```python
from build123d import *

# Parameters (mm, degrees)
BOSS_EXTRUDE1_DEPTH = 220
SHELL1_T            = -2
CUT_EXTRUDE1_DEPTH  = 321.212491043
SKETCH3_R           = 2.5
CUT_EXTRUDE2_DEPTH  = 394.612153142
SKETCH4_W           = 120
SKETCH4_H           = 120
CUT_EXTRUDE3_DEPTH  = 376.254580252
CUT_EXTRUDE4_DEPTH  = 120
FILLET1_R           = 10
CUT_EXTRUDE5_REACH  = 377.255
SKETCH6_W           = 20
SKETCH6_H           = 25
CUT_EXTRUDE6_DEPTH  = 25
FILLET2_R           = 5
SKETCH8_W           = 20
SKETCH8_H           = 52
CUT_EXTRUDE7_DEPTH  = 357.766015962
CUT_EXTRUDE8_DEPTH  = 20
FILLET3_R           = 5


with BuildPart() as part:
    # Sketch1 → Boss-Extrude1 (new body)
    with BuildSketch(Plane.XY):
        Polygon((-164.523614444, 0), (-116.335763439, -116.335763439), (0, -164.523614444), (116.335763439, -116.335763439), (164.523614444, 0), (116.335763439, 116.335763439), (0, 164.523614444), (-116.335763439, 116.335763439), align=None)
    extrude(amount=BOSS_EXTRUDE1_DEPTH)

    # Shell1
    shell1_openings = [part.faces().sort_by_distance(p)[0] for p in [
        (0, 0, 220),
        (0, 0, 0),
    ]]
    offset(amount=SHELL1_T, openings=shell1_openings, kind=Kind.INTERSECTION)

    # Sketch2 → Cut-Extrude1 (cut, through all)
    with BuildSketch(Plane.XY.offset(220)):
        Polygon((75.61693775, 182.555436661), (-82.042454152, -198.068005503), (95.714298716, -271.697263345), (253.373690618, 108.92617882), align=None)
    extrude(amount=-CUT_EXTRUDE1_DEPTH, mode=Mode.SUBTRACT)

    # Sketch3 → Cut-Extrude2 (cut, through all)
    with BuildSketch(Plane(origin=(-58.167881719, -140.429688942, 0), x_dir=(0.9238795325112961, -0.3826834323650676, 0), z_dir=(-0.3826834323650675, -0.923879532511296, 0))):
        with Locations((-12, 200)):
            Circle(SKETCH3_R)
        with Locations((-12, 140)):
            Circle(SKETCH3_R)
        with Locations((-12, 80)):
            Circle(SKETCH3_R)
    extrude(amount=-CUT_EXTRUDE2_DEPTH, mode=Mode.SUBTRACT)

    # Sketch4 → Cut-Extrude3 (cut, through all)
    with BuildSketch(Plane(origin=(-58.167881719, 140.429688942, 0), x_dir=(0.9238795325112777, 0.3826834323651116, 0), z_dir=(-0.38268343236511165, 0.9238795325112779, 0))):
        with Locations((12.039538519, -60)):
            Rectangle(SKETCH4_W, SKETCH4_H)
    extrude(amount=-CUT_EXTRUDE3_DEPTH, mode=Mode.SUBTRACT)

    # Sketch5 → Cut-Extrude4 (cut)
    with BuildSketch(Plane(origin=(0, 0, 0), x_dir=(-1, 0, 0), z_dir=(0, 0, -1))):
        Polygon((-12.944778014, 156.996927428), (-11.862385814, 159.610053358), (-13.710144879, 158.844686494), align=None)
    extrude(amount=-CUT_EXTRUDE4_DEPTH, mode=Mode.SUBTRACT)

    # Fillet1
    fillet1_edges = [part.edges().sort_by_distance(p)[0] for p in [
        (-102.094887019, 121.152135392, 120),
        (13.327461447, 157.920806961, 120),
    ]]
    fillet(fillet1_edges, radius=FILLET1_R)

    # Sketch6 → Cut-Extrude5 (cut, up to next)
    with BuildSketch(Plane(origin=(-58.167881719, 140.429688942, 0), x_dir=(0.9238795325112777, 0.3826834323651116, 0), z_dir=(-0.38268343236511165, 0.9238795325112779, 0)), mode=Mode.PRIVATE) as cut_extrude5_sk1:
        with Locations((-57.960461481, -12.5)):
            Rectangle(SKETCH6_W, SKETCH6_H)
    cut_extrude5_tool1 = extrude(cut_extrude5_sk1.sketch, amount=-CUT_EXTRUDE5_REACH, mode=Mode.PRIVATE) & part.part
    add(cut_extrude5_tool1.solids().sort_by_distance((-111.716366, 118.249181, 12.5))[0], mode=Mode.SUBTRACT)

    # Sketch7 → Cut-Extrude6 (cut)
    with BuildSketch(Plane(origin=(0, 0, 0), x_dir=(-1, 0, 0), z_dir=(0, 0, -1))):
        Polygon((117.959351739, 107.189822685), (119.04174394, 109.802948615), (119.807110804, 107.95518955), align=None)
    extrude(amount=-CUT_EXTRUDE6_DEPTH, mode=Mode.SUBTRACT)

    # Fillet2
    fillet2_edges = [part.edges().sort_by_distance(p)[0] for p in [
        (-118.883231272, 107.572506117, 25),
    ]]
    fillet(fillet2_edges, radius=FILLET2_R)

    # Sketch8 → Cut-Extrude7 (cut, through all)
    with BuildSketch(Plane(origin=(-140.429688942, 58.167881719, 0), x_dir=(0, 0, 1), z_dir=(-0.9238795325112957, 0.3826834323650681, 0))):
        with Locations((10, -40.960461481)):
            Rectangle(SKETCH8_W, SKETCH8_H)
    extrude(amount=-CUT_EXTRUDE7_DEPTH, mode=Mode.SUBTRACT)

    # Sketch9 → Cut-Extrude8 (cut)
    with BuildSketch(Plane(origin=(0, 0, 0), x_dir=(-1, 0, 0), z_dir=(0, 0, -1))):
        Polygon((159.745704114, -6.30864406), (161.593463179, -7.074010925), (162.358830044, -5.22625186), align=None)
    extrude(amount=-CUT_EXTRUDE8_DEPTH, mode=Mode.SUBTRACT)

    # Fillet3
    fillet3_edges = [part.edges().sort_by_distance(p)[0] for p in [
        (-145.230930158, 43.963534128, 20),
        (-160.669583647, -6.691327492, 20),
    ]]
    fillet(fillet3_edges, radius=FILLET3_R)


solid = part.part
```
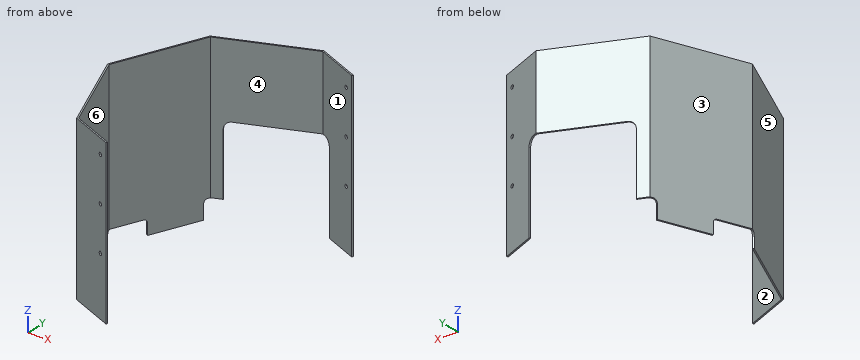
Work out the finished part from the listing and answer in its coordinate system (mm). Face numbers are marked on the shaded views. A direction names the side the tool comes from. Round coordinates to 2 decimals unless told otherwise and drop trailing zeros. Order: outer loops, then holes, each group sorted by start corner. A loop starts at its lowest first (then second) coordinate and runs counter-clockwise, first axis right, second up.
Q1. A cutting plane is placed at D-D, the plane y = -79.5. Determine the outline of the cut face in (x, z).
Solution:
outline: (-131.59, 0) - (-129.43, 0) - (-129.43, 220) - (-131.59, 220) - close
Q2. Given pin 1 Ø2 at (y, z) = (-58.5, 74) entering from -X; pin 2 Ø10 at (y, z) = (56, 167.5) entering from +X; pin 3 Ø6 at (y, z) = (-76, 87.5) entering from -X, each flat-ended and moving along its own axis, determine where each tip first touches the part or whether it passes through.
Solution:
pin 1: stops at x = -140.71
pin 2: stops at x = -137.09
pin 3: stops at x = -134.29
Q3. A cutting plane is placed at A-A, the plane z = 87. Determine the outline of the cut face in (x, y).
Solution:
outline: (-164.52, 0) - (-116.34, -116.34) - (-58.17, -140.43) - (-57.4, -138.58) - (-114.81, -114.81) - (-162.36, 0) - (-114.81, 114.81) - (-101.71, 120.23) - (-102.48, 122.08) - (-116.34, 116.34) - close; (12.94, 157) - (57.4, 138.58) - (58.17, 140.43) - (13.71, 158.84) - close
Q4. The mould has two halves that part along X. Classify the marked faces 1, 2 and 3: pulls with the +X half, pulls with the -X half, needs draft (parallel to the pull), parting line crosses it, or undercut.
Solution:
face 1: undercut
face 2: pulls with the +X half
face 3: pulls with the -X half
Q5. A cutting plane is placed at C-C, the plane z = 131.5. Determine the outline of the cut face in (x, y).
Solution:
outline: (-164.52, 0) - (-116.34, -116.34) - (-58.17, -140.43) - (-57.4, -138.58) - (-114.81, -114.81) - (-162.36, 0) - (-114.81, 114.81) - (0, 162.36) - (57.4, 138.58) - (58.17, 140.43) - (0, 164.52) - (-116.34, 116.34) - close
Q6. A cutting plane is placed at B-B, the plane x = -124.5. Determine the outline of the cut face in (y, z).
Solution:
outline: (-96.63, 0) - (-91.4, 0) - (-91.4, 220) - (-96.63, 220) - close; (91.4, 0) - (96.63, 0) - (96.63, 220) - (91.4, 220) - close
Q7. Find the intervals of material crossed by line 1 along X through (y, z) = (-97, 165); line 2 along X through (y, z) = (88.5, 118.5); line 3 along Y through (x, z) = (-117, 102.5), in increasing order.
Solution:
line 1: x = -124.34 to -122.18
line 2: x = -127.87 to -125.7
line 3: y = -114.73 to -109.51, 109.51 to 114.73
Q8. A tool of negligible diameter and unlimited length cuts with its end or side. For the marked faces 4, 5 and 6, from which of +Z, -Z, +X, -X, +Y, -Y can it reach the whole face along a straight path? Write none if from no direction.
Solution:
face 4: +Z, -Z
face 5: +Z, -Z, -X, -Y
face 6: +Z, -Z, +X
